Check sheet for the drawn part. Datum: minimum x, y, z corner. Units: mm. Coordinates: 2 decimals unless noted, no trailing zeros. Loops run counter-clockwise (first coordinate to the right, second up) from the corner with the lowest first, then second, coordinate; pieces in that order, holes last.
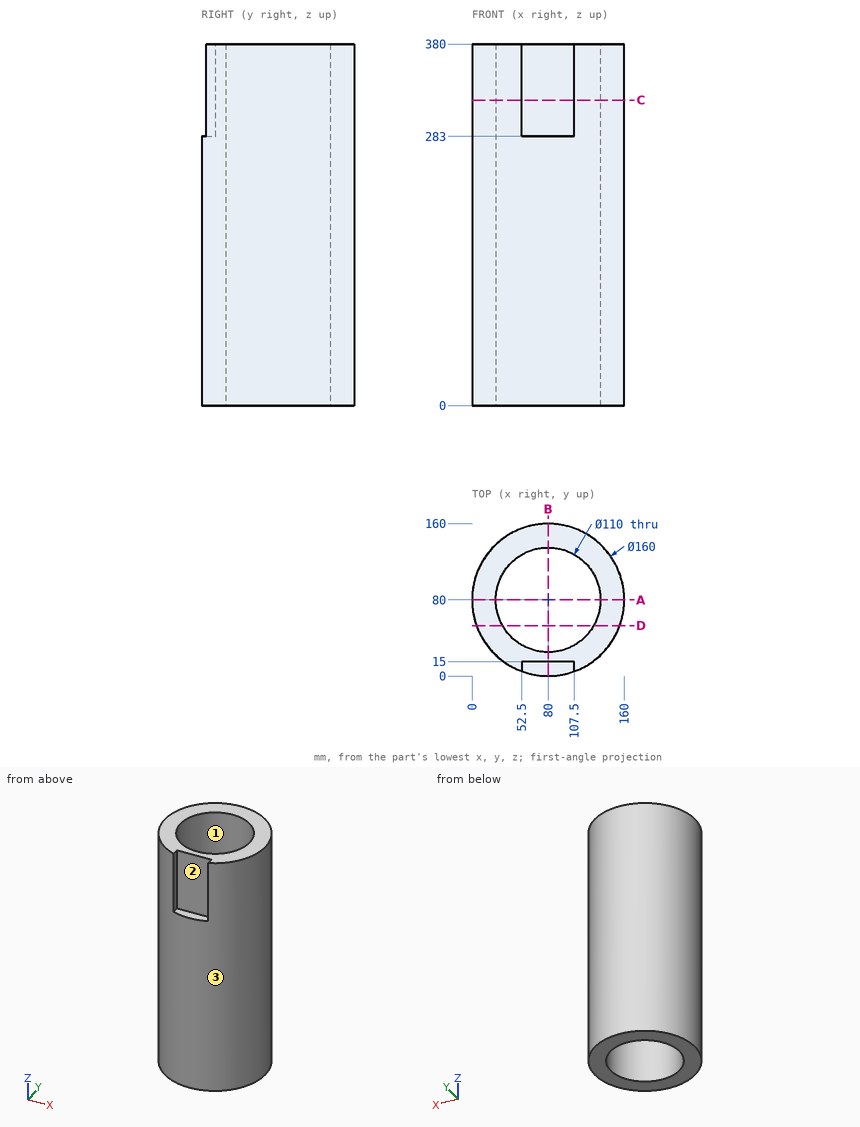
1) Depth check by flat-ended pin: pin 1 (12 mm diameter, centred on x = 72, y = 6, fed in from +Z); pin 2 (16.5 mm diameter, centred on x = 93.5, z = 320.5, fed in from -Y); pin 3 (8 mm diameter, centred on y = 11, z = 319, fed in from +X). Enter the tip coordinate at first touch or a pass-through.
Answer sheet:
pin 1: stops at z = 283
pin 2: stops at y = 15
pin 3: stops at x = 126.64
2) Scan lines: line 1 (Y direction, x = 80, z = 214); line 2 (X direction, y = 131, z = 171). Record each from-to range of solid material in increasing order.
Answer sheet:
line 1: y = 0 to 25, 135 to 160
line 2: x = 18.36 to 59.41, 100.59 to 141.64
3) Section check B-B on x = 80. Enter the section's corners in (y, z), plus the area to 3 significant figures.
Answer sheet:
outline: (0, 0) - (25, 0) - (25, 380) - (15, 380) - (15, 283) - (0, 283) - close; (135, 0) - (160, 0) - (160, 380) - (135, 380) - close
area: 17,500 mm2
4) Section check C-C on z = 321. Enter the section's corners in (x, y).
Answer sheet:
outline: (52.5, 4.88) - (52.5, 15) - (107.5, 15) - (107.5, 4.88) arc R80 ccw (long way) to start; hole circle Ø110 at (80, 80)
5) Mould release check, pull along Y, two halves, no side actions. Record for the marked faces 1, 2 and 3: +Y half, -Y half, draft (parallel to the pull), parting line (faces both ways), or undercut.
Answer sheet:
face 1: undercut
face 2: -Y half
face 3: parting line
6) Section check A-A on y = 80. Enter the section's corners in (x, z).
Answer sheet:
outline: (0, 0) - (25, 0) - (25, 380) - (0, 380) - close; (135, 0) - (160, 0) - (160, 380) - (135, 380) - close
7) Section check D-D on y = 53. Enter the section's corners in (x, z).
Answer sheet:
outline: (4.69, 0) - (32.08, 0) - (32.08, 380) - (4.69, 380) - close; (127.92, 0) - (155.31, 0) - (155.31, 380) - (127.92, 380) - close
